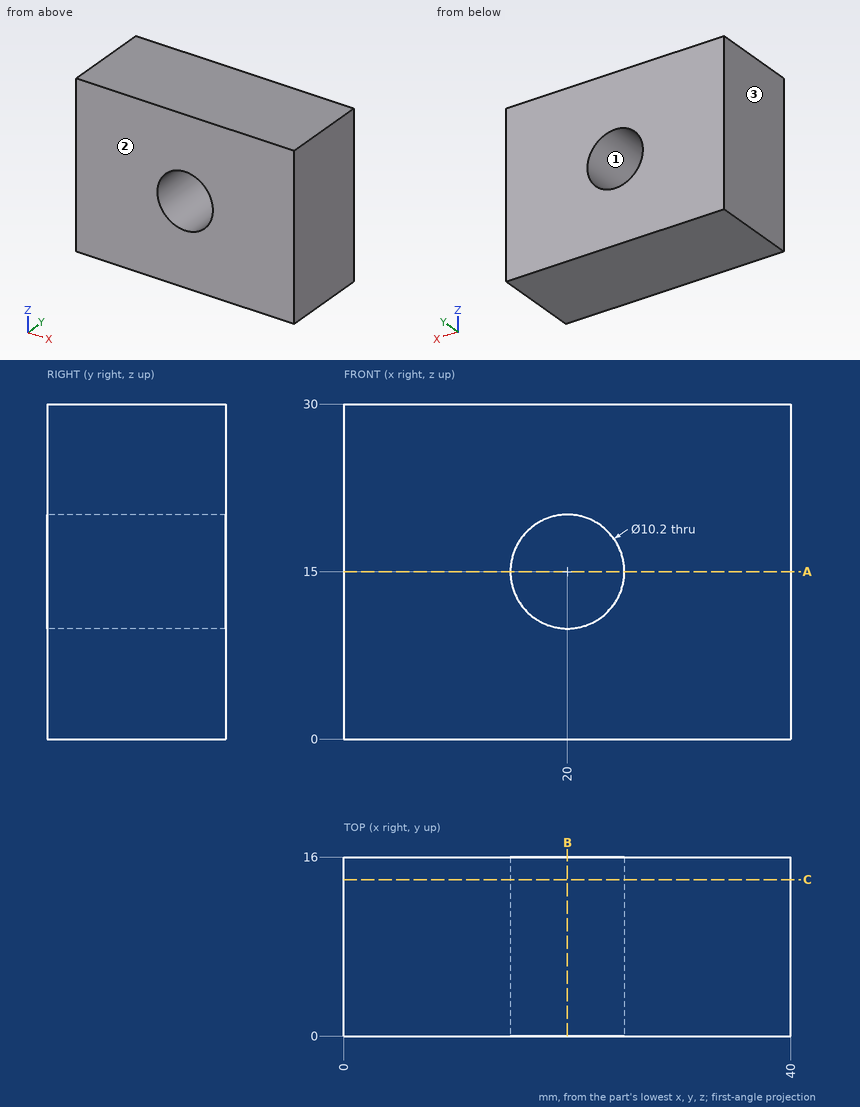
Design review of the part shown in the three views and the two pictorial views. Dimensions are in mm from the part's minimum x, y and z. Round coordinates to 2 decimals unless told otherwise and drop trailing zeros. Write each loop counter-clockwise with the first axis right and the second up, starting at its lowest first coordinate (ties: lowest second). Pieces come first, ordered by that corner, then holes.
Item 1: Wall thickness on L1, parallel to Z at x = 20, y = 12; L2, parallel to X at y = 12, z = 14.75; L3, parallel to Z at x = 17, y = 5: over which ranges is each line inside the solid? List them lowest first.
Item 2: Consider section A-A on z = 15. Give the boundary of the cut face in (x, y), and give its area (3 significant figures).
Item 3: Consider section B-B on x = 20. Give the boundary of the cut face in (y, z).
Item 4: For pin 1 Ø8 at (y, z) = (11, 22) entering from -X, flat-tipped, find the tip position at first contact; note if it passes through.
Item 5: Consider section C-C on y = 14. Give the boundary of the cut face in (x, z), and give its area (3 significant figures).
Item 6: Draft analysis for pull direction X (two halves, no side actions). For the marked faces 1, 2 and 3, state which applies: released by +X, released by -X, zero draft, split by the parting line, or undercut.
Check values:
1. L1: z = 0 to 9.9, 20.1 to 30
1. L2: x = 0 to 14.91, 25.09 to 40
1. L3: z = 0 to 10.88, 19.12 to 30
2. outline: (0, 0) - (14.9, 0) - (14.9, 16) - (0, 16) - close; (25.1, 0) - (40, 0) - (40, 16) - (25.1, 16) - close
2. area: 477 mm2
3. outline: (0, 0) - (16, 0) - (16, 9.9) - (0, 9.9) - close; (0, 20.1) - (16, 20.1) - (16, 30) - (0, 30) - close
4. pin 1: stops at x = 0
5. outline: (0, 0) - (40, 0) - (40, 30) - (0, 30) - close; hole circle Ø10.2 at (20, 15)
5. area: 1,120 mm2
6. face 1: undercut
6. face 2: zero draft
6. face 3: released by -X
